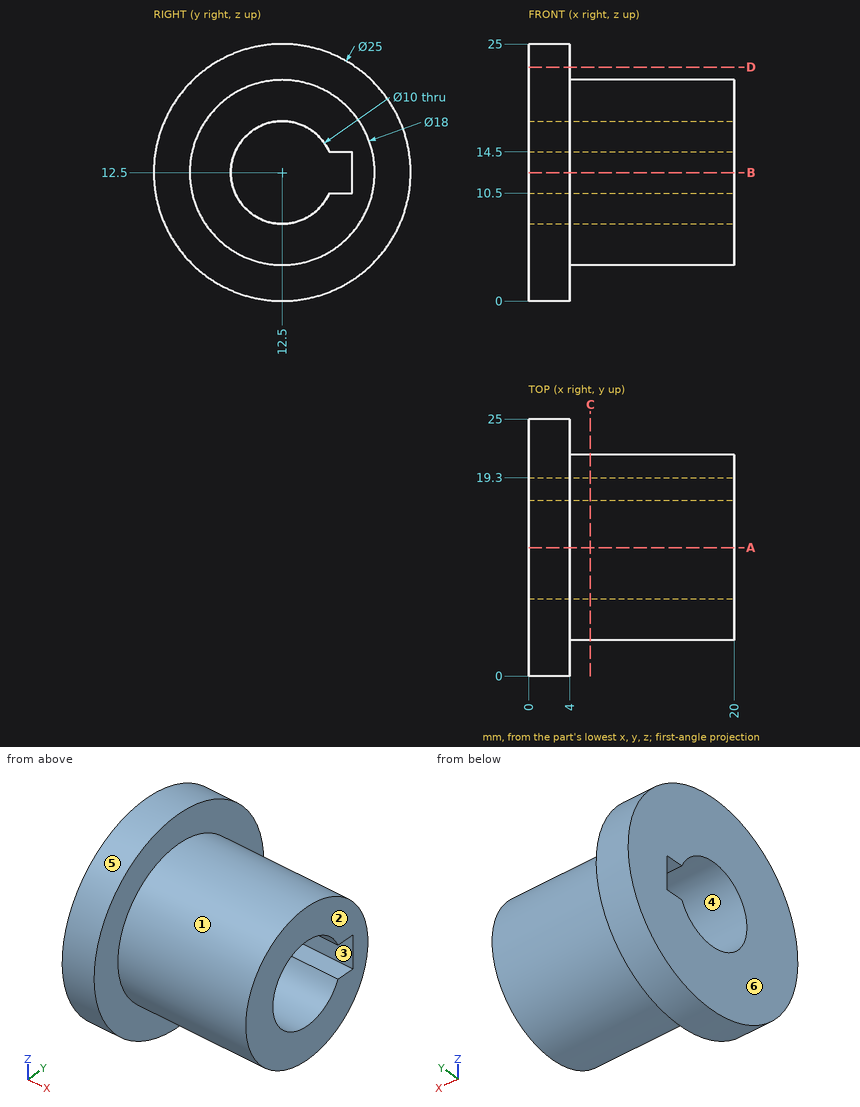
Check sheet for the drawn part. Datum: minimum x, y, z corner. Units: mm. A direction names the side the tool comes from. Round coordinates to 2 decimals unless told otherwise and drop trailing zeros. Loops run counter-clockwise (first coordinate to the right, second up) from the corner with the lowest first, then second, coordinate; pieces in that order, holes last. Notation, with made-up numbers: M 34,74 L 76,74 A21 ccw 76,108 Z; hole C 81.5,-32 d4. An arc over 180 degrees is marked long. Write each question's results on one line, items separated by ' | '.
1) Scan lines: L1, parallel to Y at x = 5.5, z = 12.5; L2, parallel to Z at x = 3.5, y = 12.75; L3, parallel to X at y = 22, z = 11.5. Record each from-to range of solid material in increasing order. Write a range as from..to.
Checks:
L1: y = 3.5..7.5, 19.3..21.5 | L2: z = 0..7.51, 17.49..25 | L3: x = 0..4
2) Section check D-D on z = 22.75. Record the boundary of the cut face in (x, y), then the cut area to 3 significant figures.
Checks:
outline: M 0,5.35 L 4,5.35 L 4,19.65 L 0,19.65 Z | area: 57.2 mm2
3) Section check B-B on z = 12.5. Record the boundary of the cut face in (x, y), then the cut area to 3 significant figures.
Checks:
outline: M 0,0 L 4,0 L 4,3.5 L 20,3.5 L 20,7.5 L 0,7.5 Z; M 0,19.3 L 20,19.3 L 20,21.5 L 4,21.5 L 4,25 L 0,25 Z | area: 152 mm2
4) Mould release check, pull along Y, two halves, no side actions. Record for the marked faces 4, 5 and 6: released by +Y, released by -Y, zero draft, split by the parting line, or undercut.
Checks:
face 4: undercut | face 5: split by the parting line | face 6: zero draft
5) Section check C-C on x = 6. Record the boundary of the cut face in (y, z).
Checks:
outline: C 12.5,12.5 d18; hole M 17.08,10.5 L 19.3,10.5 L 19.3,14.5 L 17.08,14.5 A5 ccw long Z
6) Access from +Z, -Z, +X, -X, +Y, -Y to the whole of each face (thin tool, end or side, straight path). Record for the marked faces 1, 2 and 3.
Checks:
face 1: +X | face 2: +Z, -Z, +X, +Y, -Y | face 3: +X, -X
7) Section check A-A on y = 12.5. Record the boundary of the cut face in (x, z), then the cut area to 3 significant figures.
Checks:
outline: M 0,0 L 4,0 L 4,3.5 L 20,3.5 L 20,7.5 L 0,7.5 Z; M 0,17.5 L 20,17.5 L 20,21.5 L 4,21.5 L 4,25 L 0,25 Z | area: 188 mm2
8) Gauge pin test, flat ends, axial feed: P1, Ø5, axis at x = 17.5, z = 8, coming from the +Y side; P2, Ø1.1, axis at x = 12, y = 17.5, coming from the -Z side; P3, Ø3, axis at x = 2, z = 17, coming from the -Y side; P4, Ø12, axis at y = 9.5, z = 13, coming from the -X side. Record the tip position at first contact, or that the pin passes through.
Checks:
P1: stops at y = 21.27 | P2: stops at z = 4.68 | P3: stops at y = 0.37 | P4: stops at x = 0
